Verification items for the finished model (mm, model axes). A direction names the side the tool comes from. Round coordinates to 2 decimals unless told otherwise and drop trailing zeros. Loops run counter-clockwise (first coordinate to the right, second up) from the corner with the lowest first, then second, coordinate; pieces in that order, holes last. Notation, with made-up numbers: M -8,5.25 L 44,5.25 A20 cw 44,28.25 Z; hole C 41,9.25 d5. An arc over 180 degrees is marked long. One line per item, written item: value.
from build123d import *

# Parameters (mm, degrees)
SKETCH_1_W                  = 230
SKETCH_1_H                  = 220
BOSS_EXTRUDE_1_DEPTH        = 12
CHAMFER_1_SIZE              = 20
SKETCH_11_W                 = 50
SKETCH_11_H                 = 80
CUT_EXTRUDE_1_DEPTH         = 160.590099944
M6_TAPPED_HOLE_1_D          = 5
LINEAR_PATTERN_4_COUNT      = 2
LINEAR_PATTERN_4_PITCH      = 15
LINEAR_PATTERN_5_COUNT      = 3
LINEAR_PATTERN_5_PITCH      = 50
LINEAR_PATTERN_5_COL_COUNT  = 3
LINEAR_PATTERN_5_COL_PITCH  = 50
LINEAR_PATTERN_6_COUNT      = 2
LINEAR_PATTERN_6_PITCH      = 110
LINEAR_PATTERN_6_COPY_1_D   = 5
M5_TAPPED_HOLE_2_D          = 4.2
LINEAR_PATTERN_7_COUNT      = 2
LINEAR_PATTERN_7_PITCH      = 30
LINEAR_PATTERN_7_COUNT_DIR2 = 2
LINEAR_PATTERN_7_PITCH_DIR2 = 185
LINEAR_PATTERN_8_COUNT      = 2
LINEAR_PATTERN_8_PITCH      = 139
LINEAR_PATTERN_9_COUNT      = 2
LINEAR_PATTERN_9_PITCH      = 195
M5_TAPPED_HOLE_3_D          = 4.2
LINEAR_PATTERN_10_COUNT     = 2
LINEAR_PATTERN_10_PITCH     = 60
LINEAR_PATTERN_11_COUNT     = 2
LINEAR_PATTERN_11_PITCH     = 140
LINEAR_PATTERN_12_COUNT     = 2
LINEAR_PATTERN_12_PITCH     = 170
LINEAR_PATTERN_12_COPY_1_D  = 4.2
LINEAR_PATTERN_12_COPY_2_D  = 4.2
LINEAR_PATTERN_13_COUNT     = 2
LINEAR_PATTERN_13_PITCH     = 215
LINEAR_PATTERN_13_COPY_1_D  = 5
LINEAR_PATTERN_14_COUNT     = 2
LINEAR_PATTERN_14_PITCH     = 40
LINEAR_PATTERN_14_COPY_1_D  = 5
LINEAR_PATTERN_15_COUNT     = 2
LINEAR_PATTERN_15_PITCH     = 10


with BuildPart() as part:
    # Sketch 1 → Boss-Extrude 1 (new body)
    with BuildSketch(Plane(origin=(0, 0, 0), x_dir=(0, 0, -1), z_dir=(1, 0, 0))):
        Rectangle(SKETCH_1_W, SKETCH_1_H)
    extrude(amount=BOSS_EXTRUDE_1_DEPTH)

    # Chamfer 1
    chamfer_1_edges = [part.edges().sort_by_distance(p)[0] for p in [
        (6, 110, 115),
        (6, 110, -115),
    ]]
    chamfer(chamfer_1_edges, length=CHAMFER_1_SIZE)

    # Sketch 11 → Cut-Extrude 1 (cut, through all)
    with BuildSketch(Plane.ZY):
        with Locations((50, -60)):
            Rectangle(SKETCH_11_W, SKETCH_11_H)
    extrude(amount=-CUT_EXTRUDE_1_DEPTH, mode=Mode.SUBTRACT)

    # M6 Tapped Hole 1 (through all)
    with Locations(Plane.ZY):
        with Locations((-107.5, -60)):
            m6_tapped_hole_1 = Hole(M6_TAPPED_HOLE_1_D / 2)

    # Linear Pattern 4: M6 Tapped Hole 1 ×2
    with Locations(*[(0, i * LINEAR_PATTERN_4_PITCH, 0) for i in range(1, LINEAR_PATTERN_4_COUNT)]):
        add(m6_tapped_hole_1, mode=Mode.SUBTRACT)

    # Sketch 14 → M5 Tapped Hole 1 (revolve, cut)
    with BuildSketch(Plane(origin=(6, -110, 0), x_dir=(0, 0, -1), z_dir=(1, 0, 0))):
        Polygon((0, 0), (0, 13.6618073), (2.1, 12.4), (2.1, 0), align=None)
    m5_tapped_hole_1 = revolve(axis=Axis((6, -116.35, 0), (0, 1, 0)), mode=Mode.SUBTRACT)

    # Linear Pattern 5: M5 Tapped Hole 1 ×3
    with Locations(*[(0, 0, -i * LINEAR_PATTERN_5_PITCH) for i in range(1, LINEAR_PATTERN_5_COUNT)]):
        add(m5_tapped_hole_1, mode=Mode.SUBTRACT)

    # Linear Pattern 5 col: M5 Tapped Hole 1 ×3
    with Locations(*[(0, 0, i * LINEAR_PATTERN_5_COL_PITCH) for i in range(1, LINEAR_PATTERN_5_COL_COUNT)]):
        add(m5_tapped_hole_1, mode=Mode.SUBTRACT)

    # Linear Pattern 6: M6 Tapped Hole 1 ×2
    with Locations(*[(0, 0, i * LINEAR_PATTERN_6_PITCH) for i in range(1, LINEAR_PATTERN_6_COUNT)]):
        add(m6_tapped_hole_1, mode=Mode.SUBTRACT)

    # Linear Pattern 6 copy 1 (through all)
    with Locations(Plane(origin=(0, 15, 110), x_dir=(0, 0, 1), z_dir=(-1, 0, 0))):
        with Locations((-107.5, -60)):
            Hole(LINEAR_PATTERN_6_COPY_1_D / 2)

    # M5 Tapped Hole 2 (through all)
    with Locations(Plane.ZY):
        with Locations((11.5, -91)):
            m5_tapped_hole_2 = Hole(M5_TAPPED_HOLE_2_D / 2)

    # Linear Pattern 7: M5 Tapped Hole 2 2 × 2
    with Locations(*[(0, j * LINEAR_PATTERN_7_PITCH_DIR2, -i * LINEAR_PATTERN_7_PITCH) for i in range(LINEAR_PATTERN_7_COUNT) for j in range(LINEAR_PATTERN_7_COUNT_DIR2) if (i, j) != (0, 0)]):
        add(m5_tapped_hole_2, mode=Mode.SUBTRACT)

    # Sketch 18 → Ø5.0 (5) Hole 1 (revolve, cut)
    with BuildSketch(Plane(origin=(12, -80, 97.5), x_dir=(0, 0, -1), z_dir=(0, 1, 0))):
        Polygon((0, 0), (0, 21.502151548), (2.5, 20), (2.5, 0), align=None)
    f_5_0_5_hole_1 = revolve(axis=Axis((18.35, -80, 97.5), (-1, 0, 0)), mode=Mode.SUBTRACT)

    # Linear Pattern 8: Ø5.0 (5) Hole 1 ×2
    with Locations(*[(0, i * LINEAR_PATTERN_8_PITCH, 0) for i in range(1, LINEAR_PATTERN_8_COUNT)]):
        add(f_5_0_5_hole_1, mode=Mode.SUBTRACT)

    # Linear Pattern 9: Ø5.0 (5) Hole 1 ×2
    with Locations(*[(0, 0, -i * LINEAR_PATTERN_9_PITCH) for i in range(1, LINEAR_PATTERN_9_COUNT)]):
        add(f_5_0_5_hole_1, mode=Mode.SUBTRACT)

    # Linear Pattern 9 copy 1 sketch → Linear Pattern 9 copy 1 (revolve, cut)
    with BuildSketch(Plane(origin=(12, 59, -97.5), x_dir=(0, 0, -1), z_dir=(0, 1, 0))):
        Polygon((0, 0), (0, 21.502151548), (2.5, 20), (2.5, 0), align=None)
    revolve(axis=Axis((18.35, 59, -97.5), (-1, 0, 0)), mode=Mode.SUBTRACT)

    # M5 Tapped Hole 3 (through all)
    with Locations(Plane(origin=(12, 0, 0), x_dir=(0, 0, -1), z_dir=(1, 0, 0))):
        with Locations((-82.5, -80.5)):
            m5_tapped_hole_3 = Hole(M5_TAPPED_HOLE_3_D / 2)

    # Linear Pattern 10: M5 Tapped Hole 3 ×2
    with Locations(*[(0, i * LINEAR_PATTERN_10_PITCH, 0) for i in range(1, LINEAR_PATTERN_10_COUNT)]):
        add(m5_tapped_hole_3, mode=Mode.SUBTRACT)

    # Linear Pattern 11: M5 Tapped Hole 3 ×2
    with Locations(*[(0, i * LINEAR_PATTERN_11_PITCH, 0) for i in range(1, LINEAR_PATTERN_11_COUNT)]):
        add(m5_tapped_hole_3, mode=Mode.SUBTRACT)

    # Linear Pattern 12: M5 Tapped Hole 3 ×2
    with Locations(*[(0, 0, -i * LINEAR_PATTERN_12_PITCH) for i in range(1, LINEAR_PATTERN_12_COUNT)]):
        add(m5_tapped_hole_3, mode=Mode.SUBTRACT)

    # Linear Pattern 12 copy 1 (through all)
    with Locations(Plane(origin=(12, 60, -170), x_dir=(0, 0, -1), z_dir=(1, 0, 0))):
        with Locations((-82.5, -80.5)):
            Hole(LINEAR_PATTERN_12_COPY_1_D / 2)

    # Linear Pattern 12 copy 2 (through all)
    with Locations(Plane(origin=(12, 140, -170), x_dir=(0, 0, -1), z_dir=(1, 0, 0))):
        with Locations((-82.5, -80.5)):
            Hole(LINEAR_PATTERN_12_COPY_2_D / 2)

    # Linear Pattern 13: M6 Tapped Hole 1 ×2
    with Locations(*[(0, 0, i * LINEAR_PATTERN_13_PITCH) for i in range(1, LINEAR_PATTERN_13_COUNT)]):
        add(m6_tapped_hole_1, mode=Mode.SUBTRACT)

    # Linear Pattern 13 copy 1 (through all)
    with Locations(Plane(origin=(0, 15, 215), x_dir=(0, 0, 1), z_dir=(-1, 0, 0))):
        with Locations((-107.5, -60)):
            Hole(LINEAR_PATTERN_13_COPY_1_D / 2)

    # Linear Pattern 14: M6 Tapped Hole 1 ×2
    with Locations(*[(0, 0, i * LINEAR_PATTERN_14_PITCH) for i in range(1, LINEAR_PATTERN_14_COUNT)]):
        add(m6_tapped_hole_1, mode=Mode.SUBTRACT)

    # Linear Pattern 14 copy 1 (through all)
    with Locations(Plane(origin=(0, 15, 40), x_dir=(0, 0, 1), z_dir=(-1, 0, 0))):
        with Locations((-107.5, -60)):
            Hole(LINEAR_PATTERN_14_COPY_1_D / 2)

    # Sketch 22 → M3 Tapped Hole 1 (revolve, cut)
    with BuildSketch(Plane(origin=(0, -70, -110), x_dir=(0, 0, 1), z_dir=(0, 1, 0))):
        Polygon((0, 0), (0, 8.251075774), (1.25, 7.5), (1.25, 0), align=None)
    m3_tapped_hole_1 = revolve(axis=Axis((-6.35, -70, -110), (1, 0, 0)), mode=Mode.SUBTRACT)

    # Linear Pattern 15: M3 Tapped Hole 1 ×2
    with Locations(*[(0, -i * LINEAR_PATTERN_15_PITCH, 0) for i in range(1, LINEAR_PATTERN_15_COUNT)]):
        add(m3_tapped_hole_1, mode=Mode.SUBTRACT)


solid = part.part
(1) Depth check by flat-ended pin: pin 1 Ø3 at (y, z) = (-60, -107.5) entering from -X. Enter the tip coordinate at first touch or a pass-through.
Completed:
pin 1: passes through
(2) Tool access check on faces 1 (the face through (0, 2, 2)), 2 (the face through (6, -61, 25)). Record the directions out of +Z, -Z, +X, -X, +Y, -Y that give a thin tool (end or side, any length) a straight path to the whole face; none if there is none.
Completed:
face 1: +Z, -Z, -X, +Y, -Y
face 2: +X, -X
(3) Thickness scan on L1, parallel to Y at x = 6, z = 82.5; L2, parallel to Z at x = 6, y = -103.25; L3, parallel to Z at x = 8.5, y = 59. Record the ranges inside material, lowest first. Write a range as from..to.
Completed:
L1: y = -110..-82.6, -78.4..-22.6, -18.4..57.4, 61.6..110
L2: z = -115..-102.1, -97.9..-52.1, -47.9..-2.1, 2.1..47.9, 52.1..97.9, 102.1..115
L3: z = -115..-100, -95..-89.54, -85.46..80.46, 84.54..95, 100..115
(4) Mould release check, pull along Y, two halves, no side actions. Record for faces 3 (the face through (12, 2, 2)), 4 (the face through (6, -61, 75)), 5 (the face through (6, 110, 1)): +Y half, -Y half, draft (parallel to the pull), parting line (faces both ways), or undercut.
Completed:
face 3: draft
face 4: undercut
face 5: +Y half
(5) Sectioned sample at A-A on y = -30. Enter the section's corners in (x, z).
Completed:
outline: M 0,-115 L 12,-115 L 12,25 L 0,25 Z; M 0,75 L 12,75 L 12,115 L 0,115 Z
